from build123d import *

# Parameters (mm, degrees)
SKETCH1_R           = 5.5
BOSS_EXTRUDE1_DEPTH = 1
SKETCH2_R           = 1.35
CUT_EXTRUDE1_DEPTH  = 1


with BuildPart() as part:
    # Sketch1 → Boss-Extrude1 (new body)
    with BuildSketch(Plane(origin=(0, 0, 0), x_dir=(1, 0, 0), z_dir=(0, 1, 0))):
        Polygon((7.75, -9.75), (9.75, -7.75), (9.75, 7.75), (7.75, 9.75), (-7.75, 9.75), (-9.75, 7.75), (-9.75, -7.75), (-7.75, -9.75), align=None)
        with Locations(Location((0, 0, 0), (0, 0, 270))):
            Circle(SKETCH1_R, mode=Mode.SUBTRACT)
    extrude(amount=BOSS_EXTRUDE1_DEPTH)

    # Sketch2 → Cut-Extrude1 (cut)
    with BuildSketch(Plane(origin=(0, 1, 0), x_dir=(1, 0, 0), z_dir=(0, 1, 0))):
        with Locations(Location((-7.25, 7.25, 0), (0, 0, 270))):
            Circle(SKETCH2_R)
        with Locations(Location((7.25, 7.25, 0), (0, 0, 270))):
            Circle(SKETCH2_R)
        with Locations(Location((7.25, -7.25, 0), (0, 0, 270))):
            Circle(SKETCH2_R)
        with Locations(Location((-7.25, -7.25, 0), (0, 0, 270))):
            Circle(SKETCH2_R)
    extrude(amount=-CUT_EXTRUDE1_DEPTH, mode=Mode.SUBTRACT)


solid = part.part
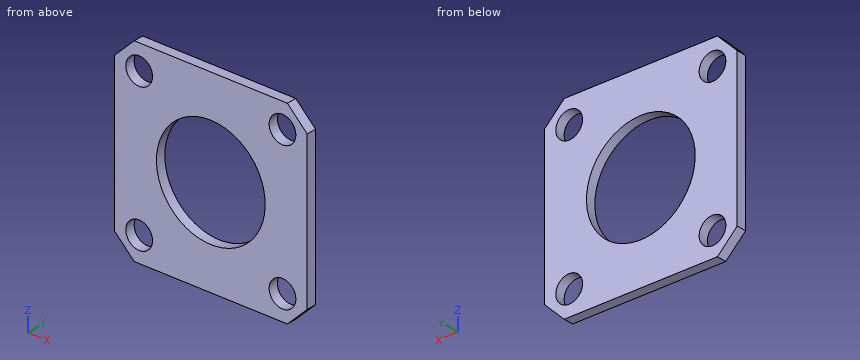
Model file for the job. Use its own axes, mm. Round coordinates to 2 decimals unless told otherwise and drop trailing zeros. Loops run counter-clockwise (first coordinate to the right, second up) from the corner with the lowest first, then second, coordinate; pieces in that order, holes last. Notation, with made-up numbers: M 29.5,-6 L 63.5,-6 A27 ccw 63.5,20 Z; hole C -7.75,17 d7. An arc over 180 degrees is marked long. One line per question, with ' | ' between items.
1) Drill centre lines: line 1 along X through (y, z) = (0.85, 7.25); line 2 along Z through (x, y) = (-8.25, 0.65); line 3 along X through (y, z) = (0.5, 0). Where is each one in solid material? Low to high.
Solved:
line 1: x = -9.75 to -8.6, -5.9 to 5.9, 8.6 to 9.75 | line 2: z = -9.25 to -8.16, -6.34 to 6.34, 8.16 to 9.25 | line 3: x = -9.75 to -5.5, 5.5 to 9.75
2) Band-saw the part on B-B (z = -6.75). Give the cut face in (x, y).
Solved:
outline: M -9.75,0 L -8.5,0 L -8.5,1 L -9.75,1 Z; M -6,0 L 6,0 L 6,1 L -6,1 Z; M 8.5,0 L 9.75,0 L 9.75,1 L 8.5,1 Z
3) Band-saw the part on A-A (x = 0). Give the cut face in (y, z), then the cut area to 3 significant figures.
Solved:
outline: M 0,-9.75 L 1,-9.75 L 1,-5.5 L 0,-5.5 Z; M 0,5.5 L 1,5.5 L 1,9.75 L 0,9.75 Z | area: 8.50 mm²
4) Band-saw the part on D-D (y = 0.45). Give the cut face in (x, z), then the cut area to 3 significant figures.
Solved:
outline: M -9.75,-7.75 L -7.75,-9.75 L 7.75,-9.75 L 9.75,-7.75 L 9.75,7.75 L 7.75,9.75 L -7.75,9.75 L -9.75,7.75 Z; hole C -7.25,-7.25 d2.7; hole C -7.25,7.25 d2.7; hole C 0,0 d11; hole C 7.25,-7.25 d2.7; hole C 7.25,7.25 d2.7 | area: 254 mm²
5) Flat gauge pins, fed straight in: pin 1 (6.5 mm diameter, centred on x = 0, z = 0, fed in from +Y); pin 2 (5 mm diameter, centred on x = -2, z = 3, fed in from -Y). Where does each tip first touch, or does it go through?
Solved:
pin 1: passes through | pin 2: stops at y = 0
6) Band-saw the part on C-C (x = -7.25). Give the cut face in (y, z).
Solved:
outline: M 0,-9.75 L 1,-9.75 L 1,-8.6 L 0,-8.6 Z; M 0,-5.9 L 1,-5.9 L 1,5.9 L 0,5.9 Z; M 0,8.6 L 1,8.6 L 1,9.75 L 0,9.75 Z
